Can you work these out from the model? Positions are in its coordinate system, mm. Face numbers are marked on the shaded views. Round coordinates to 2 decimals unless told otherwise and drop trailing zeros. Order: outer loops, then holes, each group sorted by start corner. A loop starts at its lowest first (then second) coordinate and runs counter-clockwise, first axis right, second up. Notation, with made-up numbers: M 21.25,41.25 L 70.25,41.25 A20 ccw 70.25,48.25 Z; hole C 32.25,42 d3. An arc over 180 degrees is marked long. Answer as a JSON object with one key per item and string values. Group by question number.
```python
from build123d import *

# Parameters (mm, degrees)
SKETCH1_R           = 30
SKETCH1_R_2         = 17.5
SKETCH1_R_3         = 2.5
BOSS_EXTRUDE1_DEPTH = 22


with BuildPart() as part:
    # Sketch1 → Boss-Extrude1 (new body)
    with BuildSketch(Plane.XY):
        Circle(SKETCH1_R)
        Circle(SKETCH1_R_2, mode=Mode.SUBTRACT)
        with Locations((0, 25)):
            Circle(SKETCH1_R_3, mode=Mode.SUBTRACT)
        with Locations((21.650635095, -12.5)):
            Circle(SKETCH1_R_3, mode=Mode.SUBTRACT)
        with Locations((-21.650635095, -12.5)):
            Circle(SKETCH1_R_3, mode=Mode.SUBTRACT)
    extrude(amount=BOSS_EXTRUDE1_DEPTH)


solid = part.part
```
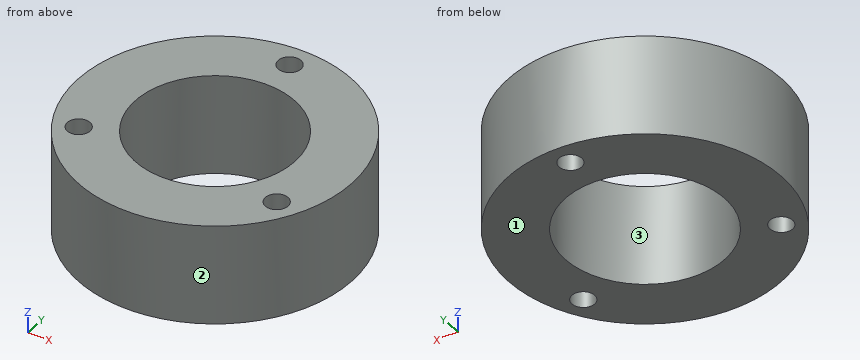
1) If we section it at D-D on z = 4.75: Write out the boundary of the cut face in (x, y).
2) If we section it at A-A on y = 0: Write out the boundary of the cut face in (x, z), plus the area to 3 significant figures.
3) I need wall thicknesses on line 1 along Y through (x, z) = (0, 5); line 2 along Y through (x, z) = (14.5, 9.75); line 3 along X through (y, z) = (-8.5, 6.75). Which ranges of each line are inside material? Lowest first, please.
4) If we section it at B-B on x = 0: Write out the boundary of the cut face in (y, z), plus the area to 3 significant figures.
5) For pin 1 (6 mm diameter, centred on y = -10.5, z = 8.5, fed in from -X); pin 2 (2 mm diameter, centred on x = 13, z = 13.5, fed in from +Y); pin 3 (6 mm diameter, centred on x = -2.5, z = 6, fed in from -Y), each with a flat end and sliding along its axis, tell me the tip position at first contact or that it passes through.
6) If we section it at C-C on x = 20.5: Write out the boundary of the cut face in (y, z).
7) We'd pull the mould along X, two halves only. Please class the marked faces 1, 2 and 3: +X half, -X half, draft (parallel to the pull), parting line (faces both ways), or undercut.
Findings:
{
 "1": {"outline": "C 0,0 d60; hole C -21.65,-12.5 d5; hole C 0,0 d35; hole C 0,25 d5; hole C 21.65,-12.5 d5"},
 "2": {"outline": "M -30,0 L -17.5,0 L -17.5,22 L -30,22 Z; M 17.5,0 L 30,0 L 30,22 L 17.5,22 Z", "area": "550 mm^2"},
 "3": {"line 1": "y = -30 to -17.5, 17.5 to 22.5, 27.5 to 30", "line 2": "y = -26.26 to -9.8, 9.8 to 26.26", "line 3": "x = -28.77 to -15.3, 15.3 to 28.77"},
 "4": {"outline": "M -30,0 L -17.5,0 L -17.5,22 L -30,22 Z; M 17.5,0 L 22.5,0 L 22.5,22 L 17.5,22 Z; M 27.5,0 L 30,0 L 30,22 L 27.5,22 Z", "area": "440 mm^2"},
 "5": {"pin 1": "stops at x = -29.05", "pin 2": "stops at y = 27.5", "pin 3": "stops at y = -30"},
 "6": {"outline": "M -21.9,0 L -14.72,0 L -14.72,22 L -21.9,22 Z; M -10.28,0 L 21.9,0 L 21.9,22 L -10.28,22 Z"},
 "7": {"face 1": "draft", "face 2": "parting line", "face 3": "undercut"}
}
